Print and shaded views of the part. All mm, measured from the part's lowest x, y and z. Coordinates: 2 decimals unless noted, no trailing zeros. Order: outer loops, then holes, each group sorted by start corner. A loop starts at its lowest first (then second) coordinate and runs counter-clockwise, first axis right, second up. Notation, with made-up numbers: M 5.25,56 L 37.25,56 A7 ccw 37.25,69 Z; hole C -7.75,9 d10. An arc over 180 degrees is marked long. Return JSON: item names as keys, results as strings.
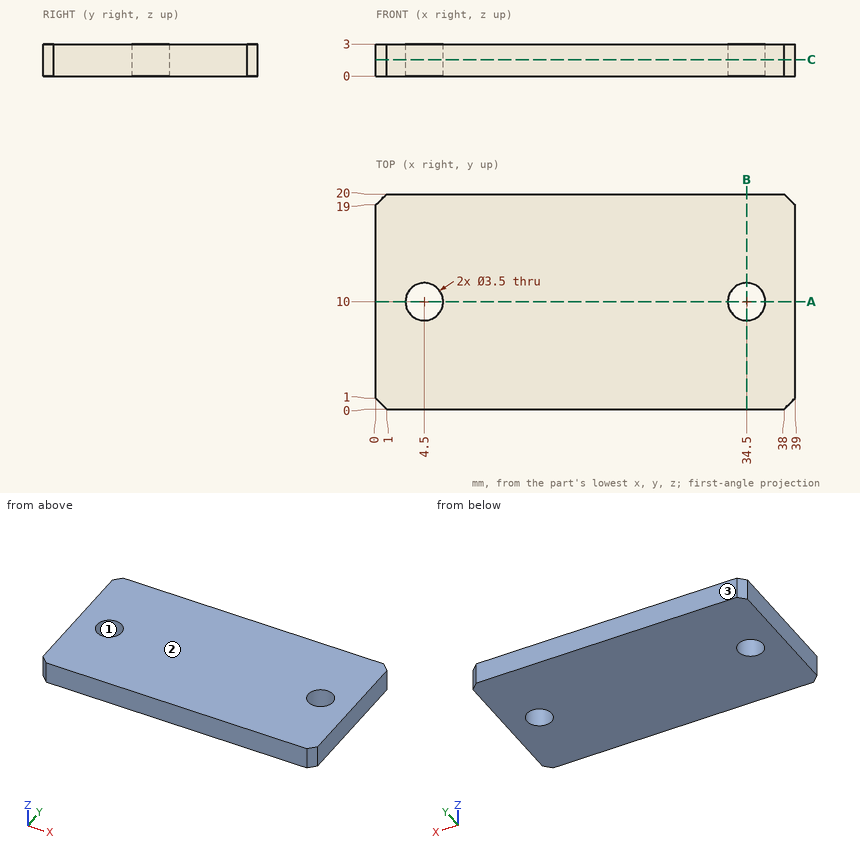
Item 1: Saw through at A-A (y = 10). Write the cut outline in (x, z).
Check result:
{"outline": "M 0,0 L 2.75,0 L 2.75,3 L 0,3 Z; M 6.25,0 L 32.75,0 L 32.75,3 L 6.25,3 Z; M 36.25,0 L 39,0 L 39,3 L 36.25,3 Z"}
Item 2: Wall check: line 1 (Y direction, x = 4.5, z = 1.7); line 2 (Y direction, x = 3.5, z = 2.3); line 3 (X direction, y = 8.75, z = 0.9). Give the ranges that are in metal, low to high.
Check result:
{"line 1": "y = 0 to 8.25, 11.75 to 20", "line 2": "y = 0 to 8.56, 11.44 to 20", "line 3": "x = 0 to 3.28, 5.72 to 33.28, 35.72 to 39"}
Item 3: Saw through at C-C (z = 1.55). Write the cut outline in (x, y).
Check result:
{"outline": "M 0,1 L 1,0 L 38,0 L 39,1 L 39,19 L 38,20 L 1,20 L 0,19 Z; hole C 4.5,10 d3.5; hole C 34.5,10 d3.5"}
Item 4: Pull direction Y, two halves, no side cores. Call the marked faces 1, 2 and 3: +Y half, -Y half, draft (parallel to the pull), parting line (faces both ways), or undercut.
Check result:
{"face 1": "undercut", "face 2": "draft", "face 3": "+Y half"}
Item 5: Saw through at B-B (x = 34.5). Write the cut outline in (y, z), and give its area (3 significant figures).
Check result:
{"outline": "M 0,0 L 8.25,0 L 8.25,3 L 0,3 Z; M 11.75,0 L 20,0 L 20,3 L 11.75,3 Z", "area": "49.5 mm2"}
